Work out the finished part from the listing and answer in its coordinate system (mm). A direction names the side the tool comes from. Give positions to 0.01 mm unless a question says otherwise; leave off trailing zeros. Loops run counter-clockwise (first coordinate to the right, second up) from the corner with the lowest first, then second, coordinate; pieces in that order, holes last. Notation, with made-up numbers: (-1.75, 30.5) - (29.25, 30.5) arc R12 ccw to (29.25, 38.5) - close; hole circle Ø6 at (10, 62). An arc over 180 degrees is marked (long way). One line per item, written item: value.
from build123d import *

# Parameters (mm, degrees)
SKETCH_1_W                   = 12
SKETCH_1_H                   = 55
EXTRUDE_1_DEPTH              = 7.5
CHAMFER_1_SIZE               = 1
HOLE_WIZARD_M6_1_D           = 6.6
HOLE_WIZARD_M6_1_CBORE_D     = 11
HOLE_WIZARD_M6_1_CBORE_DEPTH = 8
HOLE_WIZARD_M6_1_2_D         = 5


with BuildPart() as part:
    # 草图1 → 凸台-拉伸1 (new, symmetric)
    with BuildSketch(Plane(origin=(0, 0, 0), x_dir=(1, 0, 0), z_dir=(0, 1, 0))):
        Rectangle(SKETCH_1_W, SKETCH_1_H)
    extrude(amount=EXTRUDE_1_DEPTH, both=True)

    # 倒角1
    chamfer_1_edges = [part.edges().sort_by_distance(p)[0] for p in [
        (6, 0, 27.5),
        (-6, 0, 27.5),
        (-6, 0, -27.5),
        (6, 0, -27.5),
    ]]
    chamfer(chamfer_1_edges, length=CHAMFER_1_SIZE)

    # Hole Wizard M6 _1 (through all)
    with Locations(Plane(origin=(0, 7.5, 0), x_dir=(1, 0, 0), z_dir=(0, 1, 0))):
        with Locations((0, 20), (0, -20)):
            CounterBoreHole(HOLE_WIZARD_M6_1_D / 2, HOLE_WIZARD_M6_1_CBORE_D / 2, HOLE_WIZARD_M6_1_CBORE_DEPTH)

    # Hole Wizard M6 _1 2 (through all)
    with Locations(Plane.ZY.offset(6)):
        with Locations((0, 0)):
            Hole(HOLE_WIZARD_M6_1_2_D / 2)


solid = part.part
1. Section D-D (y = -4.25) is taken. Write down the section's boundary in (x, z).
Output:
outline: (-6, -26.5) - (-5, -27.5) - (5, -27.5) - (6, -26.5) - (6, 26.5) - (5, 27.5) - (-5, 27.5) - (-6, 26.5) - close; hole circle Ø6.6 at (0, -20); hole circle Ø6.6 at (0, 20)
2. Find the intervals of material crossed by line 1 along Z through (x, y) = (0, -3); line 2 along Z through (x, y) = (-1.5, -4); line 3 along X through (y, z) = (3, 20), in increasing order.
Output:
line 1: z = -27.5 to -23.3, -16.7 to 16.7, 23.3 to 27.5
line 2: z = -27.5 to -22.94, -17.06 to 17.06, 22.94 to 27.5
line 3: x = -6 to -5.5, 5.5 to 6
3. Section C-C (z = 0) is taken. Write down the section's boundary in (x, y), and give its area (3 significant figures).
Output:
outline: (-6, -7.5) - (6, -7.5) - (6, -2.5) - (-6, -2.5) - close; (-6, 2.5) - (6, 2.5) - (6, 7.5) - (-6, 7.5) - close
area: 120 mm²
4. The mould has two halves that part along X. Classify faces 3 (the cylindrical face through (-4.05, 3.56, 16.28)), 4 (the flat face through (0, 7.5, 0)), 5 (the flat face through (-5.5, 0.1, -27)), 6 (the cylindrical face through (0.72, -4.05, -16.78)): released by +X, released by -X, zero draft, split by the parting line, or undercut.
Output:
face 3: undercut
face 4: zero draft
face 5: released by -X
face 6: undercut
5. Section B-B (y = -2) is taken. Write down the section's boundary in (x, z).
Output:
outline: (-6, -26.5) - (-5, -27.5) - (5, -27.5) - (6, -26.5) - (6, -1.5) - (-6, -1.5) - close; (-6, 1.5) - (6, 1.5) - (6, 26.5) - (5, 27.5) - (-5, 27.5) - (-6, 26.5) - close; hole circle Ø6.6 at (0, -20); hole circle Ø6.6 at (0, 20)
6. Section A-A (x = 0) is taken. Write down the section's boundary in (y, z), and give its area (3 significant figures).
Output:
outline: (-7.5, -27.5) - (7.5, -27.5) - (7.5, -25.5) - (-0.5, -25.5) - (-0.5, -23.3) - (-7.5, -23.3) - close; (-7.5, -16.7) - (-0.5, -16.7) - (-0.5, -14.5) - (7.5, -14.5) - (7.5, 14.5) - (-0.5, 14.5) - (-0.5, 16.7) - (-7.5, 16.7) - close; (-7.5, 23.3) - (-0.5, 23.3) - (-0.5, 25.5) - (7.5, 25.5) - (7.5, 27.5) - (-7.5, 27.5) - close; hole circle Ø5 at (0, 0)
area: 537 mm²
7. A flat-ended cylindrical pin translates along its axis: pin 1 Ø5.5 at (x, z) = (-1, -21.5) entering from +Y. Find the tip coordinate at first contact, or state that the pin passes through.
Output:
pin 1: stops at y = -0.5
8. For faces 1 (the flat face through (0, -0.5, -16)), 2 (the flat face through (0, -7.5, 0)), determine the directions among +Z, -Z, +X, -X, +Y, -Y from which every point of the face is accessible in a straight line to the end or side of a thin tool.
Output:
face 1: +Y
face 2: +Z, -Z, +X, -X, -Y
